```python
from build123d import *

# Parameters (mm, degrees)
BASE_PROFILE_SKETCH_W = 80
BASE_PROFILE_SKETCH_H = 20
BASE_BLOCK_DEPTH      = 30
ROUND_START           = 57
ROUND_BOSS_SKETCH_R   = 15
ROUND_BOSS_SKETCH_R_2 = 7.5
ROUND_BOSS_DEPTH      = 30
INCLINED_ARM_DEPTH    = 7
ARM_WEB_SKETCH_W      = 14
ARM_WEB_SKETCH_H      = 30
ARM_WEB_DEPTH         = 7
BASE_SLOT_SKETCH_W    = 40
BASE_SLOT_SKETCH_H    = 10
BASE_SLOT_40X10_DEPTH = 138.149553408
HOLE_CUT_SKETCH_R     = 8
HOLES_16_DEPTH        = 114.004424692


with BuildPart() as part:
    # Base Profile Sketch → Base Block (new, symmetric)
    with BuildSketch(Plane.XY):
        Rectangle(BASE_PROFILE_SKETCH_W, BASE_PROFILE_SKETCH_H)
    extrude(amount=BASE_BLOCK_DEPTH, both=True)

    # Inclined Arm Sketch → Inclined Arm (add, symmetric)
    with BuildSketch(Plane(origin=(0, 0, 0), x_dir=(0, 0, -1), z_dir=(1, 0, 0))):
        Polygon((-30, 10), (38, 67), (59, 67), (59, 37), (30, -10), (30, 10), align=None)
    extrude(amount=INCLINED_ARM_DEPTH, both=True)



with BuildPart() as body_2:
    # Round Boss Sketch → Round Boss (new body)
    with BuildSketch(Plane(origin=(0, 10, 0), x_dir=(1, 0, 0), z_dir=(0, 1, 0)).offset(ROUND_START)):
        with Locations(Location((0, 74, 0), (0, 0, 270))):
            Circle(ROUND_BOSS_SKETCH_R)
        with Locations(Location((0, 74, 0), (0, 0, 270))):
            Circle(ROUND_BOSS_SKETCH_R_2, mode=Mode.SUBTRACT)
    extrude(amount=-ROUND_BOSS_DEPTH)


with BuildPart() as part_1:
    add(part.part)

    add(body_2.part)  # Arm Web merges body 2
    # Arm Web Sketch → Arm Web (add, symmetric)
    with BuildSketch(Plane(origin=(0, 0, -59), x_dir=(-1, 0, 0), z_dir=(0, 0, -1))):
        with Locations((0, 52)):
            Rectangle(ARM_WEB_SKETCH_W, ARM_WEB_SKETCH_H)
    extrude(amount=ARM_WEB_DEPTH, both=True)

    # Base Slot Sketch → Base Slot 40x10 (cut, through all)
    with BuildSketch(Plane(origin=(40, 0, 0), x_dir=(0, 0, -1), z_dir=(1, 0, 0))):
        with Locations((0, -5)):
            Rectangle(BASE_SLOT_SKETCH_W, BASE_SLOT_SKETCH_H)
    extrude(amount=-BASE_SLOT_40X10_DEPTH, mode=Mode.SUBTRACT)

    # Hole Cut Sketch → Holes Ø16 (cut, through all)
    with BuildSketch(Plane(origin=(0, 10, 0), x_dir=(1, 0, 0), z_dir=(0, 1, 0))):
        with Locations(Location((-24, 0, 0), (0, 0, 270))):
            Circle(HOLE_CUT_SKETCH_R)
        with Locations(Location((24, 0, 0), (0, 0, 270))):
            Circle(HOLE_CUT_SKETCH_R)
    extrude(amount=-HOLES_16_DEPTH, mode=Mode.SUBTRACT)


solid = part_1.part
```
Read the model definition and answer for the solid it produces. Units are mm, in the model's axes. A direction names the side the tool comes from. Round coordinates to 2 decimals unless told otherwise and drop trailing zeros. Write each loop counter-clockwise with the first axis right and the second up, starting at its lowest first coordinate (ties: lowest second). Pieces come first, ordered by that corner, then holes. Notation, with made-up numbers: (80, 57) - (139, 57) arc R15 cw to (139, 62) - close; hole circle Ø9 at (-17, 76). An arc over 180 degrees is marked (long way). One line per item, written item: value.
Q1. For a pull along Z with two mould halves and no side action, classify faces 1 (the flat face through (0.098, 13.829, -44.703)), 2 (the cylindrical face through (0.56, 52.21, -88.99)), 3 (the flat face through (4, 37, -81)), 4 (the cylindrical face through (31.932, 5.07, -1.041)) as pulls with the +Z half, pulls with the -Z half, needs draft (parallel to the pull), parting line crosses it, or undercut.
The answers:
face 1: pulls with the -Z half
face 2: parting line crosses it
face 3: needs draft
face 4: undercut
Q2. Find section B-B (x = 30.5). Determine the outline of the cut face in (y, z), and give its area (3 significant figures).
The answers:
outline: (-10, -30) - (10, -30) - (10, -4.66) - (0, -4.66) - (0, -20) - (-10, -20) - close; (-10, 20) - (0, 20) - (0, 4.66) - (10, 4.66) - (10, 30) - (-10, 30) - close
area: 707 mm2
Q3. Find section A-A (z = -74). Determine the outline of the cut face in (x, y), and give its area (3 significant figures).
The answers:
outline: (-15, 37) - (-7.5, 37) - (-7.5, 67) - (-15, 67) - close; (7.5, 37) - (15, 37) - (15, 67) - (7.5, 67) - close
area: 450 mm2
Q4. Straight lines are drawn through the part: line 1 (X direction, y = 2.5, z = 0); line 2 (X direction, y = 47, z = -74); line 3 (Y direction, x = -29.5, z = -17.5). For each, find the intervals that lie inside material, in ascending order. Write a range as from..to.
The answers:
line 1: x = -40..-32, -16..16, 32..40
line 2: x = -15..-7.5, 7.5..15
line 3: y = 0..10
Q5. Each of these flat-tipped pins is pushed along its axis until it touches: P1, Ø10, axis at y = 57.5, z = -40.5, coming from the +X side; P2, Ø21, axis at x = -24, z = 0, coming from the +Y side; P3, Ø14.5, axis at x = 24, z = 0, coming from the +Y side; P4, Ø6, axis at x = 28, y = -3, coming from the -Z side. Where does it stop, or does it pass through?
The answers:
P1: stops at x = 7
P2: stops at y = 10
P3: passes through
P4: stops at z = -30
Q6. Find section C-C (y = 41). Determine the outline of the cut face in (x, z).
The answers:
outline: (-7, -60.73) arc R15 ccw (long way) to (7, -60.73) - (7, -6.98) - (-7, -6.98) - close; hole circle Ø15 at (0, -74)
Q7. Which of the six approach directions +Z, -Z, +X, -X, +Y, -Y give full straight-line access (tool end or side, diameter ignored) to faces 5 (the flat face through (-16, 10, 7)), 6 (the flat face through (-24, 0, -30)), 7 (the flat face through (23, 0, -30)), 8 (the flat face through (1, -5, 20)), 9 (the flat face through (0, 67, -63))?
The answers:
face 5: +Z, -Z, -X, +Y
face 6: -Z, -X, +Y, -Y
face 7: -Z, +X, +Y, -Y
face 8: +X, -X, -Y
face 9: +Z, -Z, +X, -X, +Y
Q8. Find section D-D (x = -34.5). Determine the outline of the cut face in (y, z), and give its area (3 significant figures).
The answers:
outline: (-10, -30) - (10, -30) - (10, 30) - (-10, 30) - (-10, 20) - (0, 20) - (0, -20) - (-10, -20) - close
area: 800 mm2
